Geometry: final body of the model. Coordinates: model frame, mm. A direction names the side the tool comes from. Coordinates: 2 decimals unless noted, no trailing zeros. Loops run counter-clockwise (first coordinate to the right, second up) from the corner with the lowest first, then second, coordinate; pieces in that order, holes last. Notation, with made-up numbers: (19, -21.75) - (63, -21.75) arc R26 ccw to (63, 1.25) - close; hole circle Ø6 at (64.25, 13.25). An arc over 180 degrees is marked (long way). Answer in a Markdown table with one row per item.
from build123d import *

# Parameters (mm, degrees)
SKETCH1_W           = 500
SKETCH1_H           = 24
BOSS_EXTRUDE1_DEPTH = 400
SKETCH2_W           = 430
SKETCH2_H           = 8
CUT_EXTRUDE1_DEPTH  = 641.762046317
SKETCH3_W           = 544.957019416
SKETCH3_H           = 0.5
CUT_EXTRUDE2_DEPTH  = 641.762046317
SKETCH12_W          = 569.007892772
SKETCH12_H          = 39.328779912
CUT_EXTRUDE3_DEPTH  = 641.762046317
SKETCH16_W          = 24
SKETCH16_H          = 60
SKETCH16_W_2        = 20
CUT_EXTRUDE4_DEPTH  = 2
FILLET1_R           = 5


with BuildPart() as part:
    # Sketch1 → Boss-Extrude1 (new body)
    with BuildSketch(Plane.XY):
        with Locations((250, 12)):
            Rectangle(SKETCH1_W, SKETCH1_H)
    extrude(amount=-BOSS_EXTRUDE1_DEPTH)

    # Sketch2 → Cut-Extrude1 (cut, through all)
    with BuildSketch(Plane.XY):
        with Locations((250, 12)):
            Rectangle(SKETCH2_W, SKETCH2_H)
    extrude(amount=-CUT_EXTRUDE1_DEPTH, mode=Mode.SUBTRACT)

    # Sketch3 → Cut-Extrude2 (cut, through all)
    with BuildSketch(Plane.XY):
        with Locations((250, 12)):
            Rectangle(SKETCH3_W, SKETCH3_H)
    extrude(amount=-CUT_EXTRUDE2_DEPTH, mode=Mode.SUBTRACT)


with BuildPart() as cut_extrude2_piece_1:
    # of the separate pieces the step leaves, piece 1, a body of its own (cut_extrude2_pieces)
    add(part.part.solids().sort_by_distance((0, 0, 0))[0])

    # Sketch16 → Cut-Extrude4 (cut)
    with BuildSketch(Plane(origin=(0, 11.75, 0), x_dir=(1, 0, 0), z_dir=(0, 1, 0))):
        with Locations((12, 330)):
            Rectangle(SKETCH16_W, SKETCH16_H)
        with Locations((12, 70)):
            Rectangle(SKETCH16_W, SKETCH16_H)
        with Locations((10, 200)):
            Rectangle(SKETCH16_W_2, SKETCH16_H)
    extrude(amount=-CUT_EXTRUDE4_DEPTH, mode=Mode.SUBTRACT)

    # Fillet1
    fillet1_edges = [cut_extrude2_piece_1.edges().sort_by_distance(p)[0] for p in [
        (24, 10.75, -360),
        (24, 10.75, -300),
        (24, 10.75, -40),
        (24, 10.75, -100),
        (20, 10.75, -230),
        (20, 10.75, -170),
    ]]
    fillet(fillet1_edges, radius=FILLET1_R)


with BuildPart() as cut_extrude2_piece_2:
    # of the separate pieces the step leaves, piece 2, a body of its own (cut_extrude2_pieces)
    add(part.part.solids().sort_by_distance((0, 24, 0))[0])

    # Sketch12 → Cut-Extrude3 (cut, through all)
    with BuildSketch(Plane.XY):
        with Locations((265.175540793, 31.664389956)):
            Rectangle(SKETCH12_W, SKETCH12_H)
    extrude(amount=-CUT_EXTRUDE3_DEPTH, mode=Mode.SUBTRACT)


solid = cut_extrude2_piece_1.part
(1) Access query for faces 4 (the face through (12, 9.75, -330)), 5 (the face through (247, 5, 0)). Directions: +Z, -Z, +X, -X, +Y, -Y. A direction counts if a zero-diameter tool reaches every point of the face in a straight line with its end or side. Return the directions, or none.
Verdict:
| item | result |
|---|---|
| face 4 | -X, +Y |
| face 5 | +Z, +X, -X, +Y, -Y |
(2) Cut plane C-C on z = -323. Output: boundary loops of the cut face in (x, y), then the cut area to 3 significant figures.
Verdict:
| item | result |
|---|---|
| outline | (0, 0) - (500, 0) - (500, 11.75) - (465, 11.75) - (465, 8) - (35, 8) - (35, 11.75) - (24, 11.75) - (24, 9.75) - (0, 9.75) - close |
| area | 4,210 mm² |
(3) First-contact query: pin 1 Ø1.6 at (y, z) = (11, -202) entering from -X; pin 2 Ø6 at (x, z) = (7, -215) entering from +Y; pin 3 Ø0.6 at (y, z) = (11, -339) entering from -X. Flat tips, straight axial feed; report the tip coordinate or a pass-through.
Verdict:
| item | result |
|---|---|
| pin 1 | stops at x = 20 |
| pin 2 | stops at y = 9.75 |
| pin 3 | stops at x = 24 |
(4) Cut plane B-B on x = 168. Output: boundary loops of the cut face in (y, z).
Verdict:
| item | result |
|---|---|
| outline | (0, -400) - (8, -400) - (8, 0) - (0, 0) - close |
(5) Ray query, probe 1 along X at (y, z) = (11, -87); probe 2 along X at (y, z) = (8.75, -110.5); probe 3 along Y at (x, z) = (171, -152.5). Return the intervals inside material, ascending.
Verdict:
| item | result |
|---|---|
| probe 1 | x = 24 to 35, 465 to 500 |
| probe 2 | x = 0 to 35, 465 to 500 |
| probe 3 | y = 0 to 8 |
(6) Pull-direction query (X, two-part tool) for faces 1 (the face through (247, 8, -197)), 2 (the face through (0, 6, -197)), 3 (the face through (12, 9.75, -70)); classes: pulls with the +X half, pulls with the -X half, needs draft (parallel to the pull), parting line crosses it, or undercut.
Verdict:
| item | result |
|---|---|
| face 1 | undercut |
| face 2 | pulls with the -X half |
| face 3 | needs draft |
(7) Cut plane A-A on z = -139.5. Output: boundary loops of the cut face in (x, y), then the cut area to 3 significant figures.
Verdict:
| item | result |
|---|---|
| outline | (0, 0) - (500, 0) - (500, 11.75) - (465, 11.75) - (465, 8) - (35, 8) - (35, 11.75) - (0, 11.75) - close |
| area | 4,260 mm² |
